Input: part model. Units: mm. Frame: model coordinates. Give positions to 0.01 mm unless a question says otherwise; leave off trailing zeros. Loops run counter-clockwise (first coordinate to the right, second up) from the corner with the lowest first, then second, coordinate; pieces in that order, holes last. Notation, with made-up numbers: (0, 65) -> (46, 65) arc R10 ccw to (46, 73) -> close; hole circle Ø9 at (-30.75, 31.5). An arc over 180 degrees is marked (long way). One line per question, with ' | ' between items.
from build123d import *

# Parameters (mm, degrees)
SKETCH_1_W          = 106
SKETCH_1_H          = 70
EXTRUDE_1_DEPTH     = 2.5
SKETCH_2_R          = 2.1
CUT_EXTRUDE_1_DEPTH = 64.710281745
FILLET_1_R          = 3


with BuildPart() as part:
    # 草图1 → 凸台-拉伸1 (new, symmetric)
    with BuildSketch(Plane.XY):
        Rectangle(SKETCH_1_W, SKETCH_1_H)
    extrude(amount=EXTRUDE_1_DEPTH, both=True)

    # 草图2 → 切除-拉伸1 (cut, through all)
    with BuildSketch(Plane.XY.offset(2.5)):
        with Locations((-43, 25)):
            Circle(SKETCH_2_R)
        with Locations(Location((43, 25, 0), (0, 0, 180))):
            Circle(SKETCH_2_R)
        with Locations((43, -25)):
            Circle(SKETCH_2_R)
        with Locations(Location((-43, -25, 0), (0, 0, 180))):
            Circle(SKETCH_2_R)
    extrude(amount=-CUT_EXTRUDE_1_DEPTH, mode=Mode.SUBTRACT)

    # 圆角1
    fillet_1_edges = [part.edges().sort_by_distance(p)[0] for p in [
        (53, -35, 0),
        (-53, -35, 0),
        (-53, 35, 0),
        (53, 35, 0),
    ]]
    fillet(fillet_1_edges, radius=FILLET_1_R)


solid = part.part
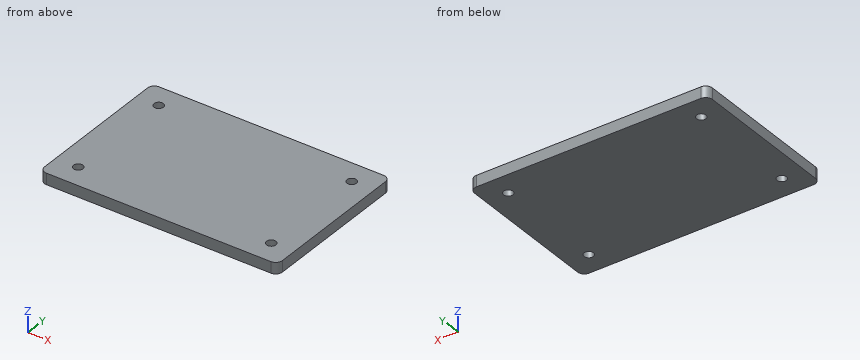
1. Pin query (flat end, axial travel): P1, Ø4, axis at x = 43, y = -25, coming from the +Z side. Return the tip coordinate at first contact, or that it passes through.
Determined:
P1: passes through
2. Section query B-B (x = -43). Output: boundary loops of the cut face in (y, z), then the cut area to 3 significant figures.
Determined:
outline: (-35, -2.5) -> (-27.1, -2.5) -> (-27.1, 2.5) -> (-35, 2.5) -> close; (-22.9, -2.5) -> (22.9, -2.5) -> (22.9, 2.5) -> (-22.9, 2.5) -> close; (27.1, -2.5) -> (35, -2.5) -> (35, 2.5) -> (27.1, 2.5) -> close | area: 308 mm2
3. Ray query, line 1 along Y through (x, z) = (-43, 0.15); line 2 along Y through (x, z) = (44, -2.2). Return the intervals inside material, ascending. Write a range as from..to.
Determined:
line 1: y = -35..-27.1, -22.9..22.9, 27.1..35 | line 2: y = -35..-26.85, -23.15..23.15, 26.85..35
4. Section query A-A (y = 25). Output: boundary loops of the cut face in (x, z), then the cut area to 3 significant figures.
Determined:
outline: (-53, -2.5) -> (-45.1, -2.5) -> (-45.1, 2.5) -> (-53, 2.5) -> close; (-40.9, -2.5) -> (40.9, -2.5) -> (40.9, 2.5) -> (-40.9, 2.5) -> close; (45.1, -2.5) -> (53, -2.5) -> (53, 2.5) -> (45.1, 2.5) -> close | area: 488 mm2
